from build123d import *

# Parameters (mm, degrees)
SKETCH_1_W                   = 120
SKETCH_1_H                   = 65
EXTRUDE_1_DEPTH              = 10
CHAMFER_1_SIZE               = 2
SKETCH_2_W                   = 120
SKETCH_2_H                   = 65
EXTRUDE_2_DEPTH              = 30
SKETCH_3_R                   = 10
CUT_EXTRUDE_1_DEPTH          = 2
HOLE_WIZARD_M6_1_D           = 6.6
HOLE_WIZARD_M6_1_CBORE_D     = 13
HOLE_WIZARD_M6_1_CBORE_DEPTH = 35
SKETCH_6_W                   = 60
SKETCH_6_H                   = 400
EXTRUDE_3_DEPTH              = 30
SKETCH_7_W                   = 60
SKETCH_7_H                   = 65
CUT_EXTRUDE_2_DEPTH          = 40


with BuildPart() as part:
    # 草图1 → 凸台-拉伸1 (new body)
    with BuildSketch(Plane.XY):
        Rectangle(SKETCH_1_W, SKETCH_1_H)
    extrude(amount=EXTRUDE_1_DEPTH)

    # 倒角1
    chamfer_1_edges = [part.edges().sort_by_distance(p)[0] for p in [
        (-60, 0, 10),
        (0, -32.5, 10),
        (60, 0, 10),
        (0, 32.5, 10),
    ]]
    chamfer(chamfer_1_edges, length=CHAMFER_1_SIZE)

    # 草图2 → 凸台-拉伸2 (add)
    with BuildSketch(Plane.XY.offset(10)):
        Rectangle(SKETCH_2_W, SKETCH_2_H)
    extrude(amount=EXTRUDE_2_DEPTH)

    # 草图3 → 切除-拉伸1 (cut)
    with BuildSketch(Plane(origin=(0, 0, 0), x_dir=(-1, 0, 0), z_dir=(0, 0, -1))):
        with Locations((-32.5, 0)):
            Circle(SKETCH_3_R)
    extrude(amount=-CUT_EXTRUDE_1_DEPTH, mode=Mode.SUBTRACT)

    # M6 六角头螺栓的柱形沉头孔1 (through all)
    with Locations(Plane.XY.offset(40)):
        with Locations((32.5, 0)):
            CounterBoreHole(HOLE_WIZARD_M6_1_D / 2, HOLE_WIZARD_M6_1_CBORE_D / 2, HOLE_WIZARD_M6_1_CBORE_DEPTH)

    # 草图6 → 凸台-拉伸3 (add)
    with BuildSketch(Plane.XY.offset(40)):
        with Locations((-30, 0)):
            Rectangle(SKETCH_6_W, SKETCH_6_H)
    extrude(amount=-EXTRUDE_3_DEPTH)

    # 草图7 → 切除-拉伸2 (cut)
    with BuildSketch(Plane.XY.offset(40)):
        with Locations((30, 0)):
            Rectangle(SKETCH_7_W, SKETCH_7_H)
    extrude(amount=-CUT_EXTRUDE_2_DEPTH, mode=Mode.SUBTRACT)


solid = part.part
Build history of the part. All positions in model axes, mm. A direction names the side the tool comes from. Coordinates: 2 decimals unless noted, no trailing zeros. Order: outer loops, then holes, each group sorted by start corner. A loop starts at its lowest first (then second) coordinate and runs counter-clockwise, first axis right, second up. Notation, with made-up numbers: (21.5, 21) -> (47.5, 21) arc R21 cw to (47.5, 27) -> close; hole circle Ø4 at (15, -17.5). An arc over 180 degrees is marked (long way). One line per item, written item: value.
(1) Slice it at A-A, the plane x = -36. List the corners of the cut face in (y, z).
Checked values:
outline: (-200, 10) -> (-30.5, 10) -> (-32.5, 8) -> (-32.5, 0) -> (32.5, 0) -> (32.5, 8) -> (30.5, 10) -> (200, 10) -> (200, 40) -> (-200, 40) -> close
(2) Tool access for faces 1 (the flat face through (-30, 32.5, 4)), 2 (the flat face through (-30, -32.5, 4)), 3 (the flat face through (-30, 0, 0)): list every direction of +Z, -Z, +X, -X, +Y, -Y with a clear straight run to the whole face (end or side of a thin tool).
Checked values:
face 1: -Z, +X, -X, +Y
face 2: -Z, +X, -X, -Y
face 3: -Z, +X, -X, +Y, -Y
(3) Drop flat-ended pins along their axis: pin 1 Ø3 at (x, y) = (-15.5, 6.5) entering from -Z; pin 2 Ø1 at (x, y) = (-25, 52.5) entering from -Z; pin 3 Ø9 at (x, z) = (-36.5, 4) entering from +Y; pin 4 Ø9 at (x, z) = (-27.5, 5) entering from -Y. Give the stop position or say it passes through.
Checked values:
pin 1: z = 0
pin 2: z = 10
pin 3: y = 32.5
pin 4: y = -32.5
(4) Probe line 1 (Z direction, x = -56, y = -58); line 2 (Y direction, x = -3, z = 8). List the from-to ranges inside material, lowest first. Write a range as [from, to].
Checked values:
line 1: [10, 40]
line 2: [-32.5, 32.5]
(5) Slice it at B-B, the plane y = 73. List the corners of the cut face in (x, z).
Checked values:
outline: (-60, 10) -> (0, 10) -> (0, 40) -> (-60, 40) -> close
